Geometry check sheet. Reference: the model listing, model coordinates, mm. Round coordinates to 2 decimals unless told otherwise and drop trailing zeros. Write each loop counter-clockwise with the first axis right and the second up, starting at its lowest first coordinate (ties: lowest second). Pieces come first, ordered by that corner, then holes.
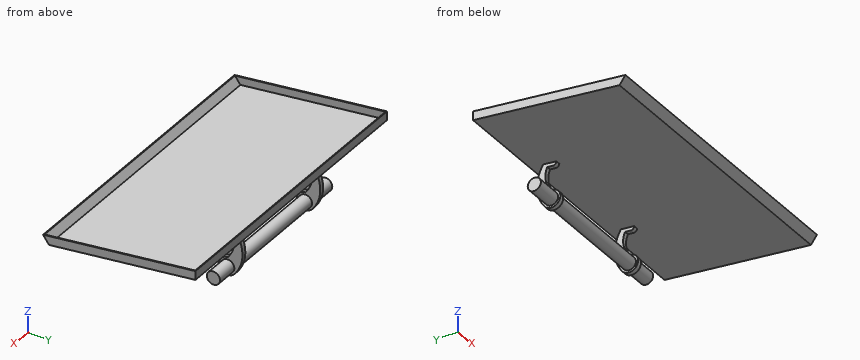
from build123d import *

# Parameters (mm, degrees)
BOSS_EXTRUDE1_DEPTH = 2
BOSS_EXTRUDE2_DEPTH = 661
BOSS_EXTRUDE3_DEPTH = 2
SKETCH4_R           = 15
BOSS_EXTRUDE4_DEPTH = 10
LPATTERN1_COUNT     = 2
LPATTERN1_PITCH     = 270
SKETCH5_R           = 15
BOSS_EXTRUDE5_DEPTH = 340
SKETCH6_R           = 15
BOSS_EXTRUDE6_DEPTH = 50


with BuildPart() as part:
    # Sketch1 → Boss-Extrude1 (new body)
    with BuildSketch(Plane(origin=(0, 0, 0), x_dir=(0, 0, -1), z_dir=(1, 0, 0))):
        Polygon((0, 0), (-20, 0), (21.83385642, -347.490904136), (40.177865273, -333.735493803), align=None)
    extrude(amount=BOSS_EXTRUDE1_DEPTH)

    # Sketch2 → Boss-Extrude2 (add)
    with BuildSketch(Plane.ZY):
        Polygon((0, 0), (20, 0), (19.759223301, -2), (1.773664518, -2), (-38.054187031, -332.828121742), (-21.557824554, -345.198058798), (-21.83385642, -347.490904136), (-40.177865273, -333.735493803), align=None)
    extrude(amount=BOSS_EXTRUDE2_DEPTH)

    # Sketch3 → Boss-Extrude3 (add)
    with BuildSketch(Plane.ZY.offset(661)):
        Polygon((20, 0), (0, 0), (-40.177865273, -333.735493803), (-21.83385642, -347.490904136), align=None)
    extrude(amount=BOSS_EXTRUDE3_DEPTH)

    # Sketch4 → Boss-Extrude4 (add)
    with BuildSketch(Plane(origin=(-195.5, 0, 0), x_dir=(0, 0, -1), z_dir=(1, 0, 0))):
        with BuildLine():
            Line((3.607407095, -29.964752484), (7.274393684, -60.424399152))
            Line((7.274393684, -60.424399152), (8.267224839, -60.304873847))
            ThreePointArc((8.267224839, -60.304873847), (12.936431276, -57.677699188), (14.380365793, -52.518378636))
            Line((14.380365793, -52.518378636), (12.826139197, -39.608270621))
            add(Edge.make_bspline(
                [(12.826139197, -39.608270621), (40.794384715, -27.323032004), (68.669426918, -49.466360803)],
                knots=[0, 0, 0, 1, 1, 1], degree=2))
            ThreePointArc((68.669426918, -49.466360803), (97.431993806, -67.44460937), (100.991169072, -33.712800243))
            add(Edge.make_bspline(
                [(3.607407095, -29.964752484), (33.423426205, -12.412570219), (69.250962672, -8.887006882), (100.991169072, -33.712800243)],
                knots=[0, 0, 0, 0, 1, 1, 1, 1], degree=3))
        make_face()
        with Locations((88.669426918, -49.466360803)):
            Circle(SKETCH4_R, mode=Mode.SUBTRACT)
    boss_extrude4 = extrude(amount=BOSS_EXTRUDE4_DEPTH)

    # LPattern1: Boss-Extrude4 ×2
    with Locations(*[(-i * LPATTERN1_PITCH, 0, 0) for i in range(1, LPATTERN1_COUNT)]):
        add(boss_extrude4)



with BuildPart() as body_2:
    # Sketch5 → Boss-Extrude5 (new body)
    with BuildSketch(Plane(origin=(-185.5, 0, 0), x_dir=(0, 0, -1), z_dir=(1, 0, 0))):
        with Locations((88.669426918, -49.466360803)):
            Circle(SKETCH5_R)
    extrude(amount=-BOSS_EXTRUDE5_DEPTH)


with BuildPart() as part_1:
    add(part.part)

    add(body_2.part)  # Boss-Extrude6 merges body 2
    # Sketch6 → Boss-Extrude6 (add)
    with BuildSketch(Plane(origin=(-185.5, 0, 0), x_dir=(0, 0, -1), z_dir=(1, 0, 0))):
        with Locations((88.669426918, -49.466360803)):
            Circle(SKETCH6_R)
    extrude(amount=BOSS_EXTRUDE6_DEPTH)


solid = part_1.part
1. Scan lines: line 1 along X through (y, z) = (-275, -29); line 2 along Y through (x, z) = (-344.5, 10); line 3 along X through (y, z) = (-26.5, -55). Record each from-to range of solid material in increasing order.
2. Depth check by flat-ended pin: pin 1 Ø1 at (x, y) = (-159.5, -53.5) entering from -Z; pin 2 Ø16 at (y, z) = (-30.5, -38.5) entering from -X; pin 3 Ø9 at (y, z) = (-52.5, -89) entering from -X. Enter the tip coordinate at first touch or a pass-through.
3. Section check B-B (x = -68). Record the cut outline in (y, z), plus the area to 3 significant figures.
4. Section check A-A (x = -228). Record the cut outline in (y, z).
Results below:
1. line 1: x = -663 to -661, 0 to 2
1. line 2: y = -2 to 0
1. line 3: x = -465.5 to -455.5, -195.5 to -185.5
2. pin 1: stops at z = -103.25
2. pin 2: stops at x = -465.5
2. pin 3: stops at x = -525.5
3. outline: (-347.49, -21.83) - (-333.74, -40.18) - (0, 0) - (0, 20) - (-2, 19.76) - (-2, 1.77) - (-332.83, -38.05) - (-345.2, -21.56) - close
3. area: 751 mm2
4. outline: (-347.49, -21.83) - (-333.74, -40.18) - (0, 0) - (0, 20) - (-2, 19.76) - (-2, 1.77) - (-332.83, -38.05) - (-345.2, -21.56) - close; circle Ø30 at (-49.47, -88.67)
